```python
from build123d import *

# Parameters (mm, degrees)
BRICK_BODY_PROFILE_W         = 31.8
BRICK_BODY_PROFILE_H         = 15.8
BRICK_BODY_DEPTH             = 9.6
STUDS_PROFILE_2X4_4_8_R      = 2.4
STUDS_8X_4_8_DEPTH           = 1.8
UNDERSIDE_CAVITY_DEPTH       = 22.099289088
UNDERSIDE_CAVITY_DEPTH_BACK  = 7.5
UNDERSIDE_CAVITY_PROFILE_R   = 3.25
UNDERSIDE_CAVITY_PROFILE_R_2 = 2.65


with BuildPart() as part:
    # Brick Body Profile → Brick Body (new body)
    with BuildSketch(Plane.XY):
        Rectangle(BRICK_BODY_PROFILE_W, BRICK_BODY_PROFILE_H)
    extrude(amount=BRICK_BODY_DEPTH)

    # Studs Profile 2x4 Ø4.8 → Studs 8xØ4.8 (add)
    with BuildSketch(Plane.XY.offset(9.6)):
        with Locations((-12, 4)):
            Circle(STUDS_PROFILE_2X4_4_8_R)
        with Locations((-4, 4)):
            Circle(STUDS_PROFILE_2X4_4_8_R)
        with Locations((4, 4)):
            Circle(STUDS_PROFILE_2X4_4_8_R)
        with Locations((12, 4)):
            Circle(STUDS_PROFILE_2X4_4_8_R)
        with Locations(Location((12, -4, 0), (0, 0, 180))):
            Circle(STUDS_PROFILE_2X4_4_8_R)
        with Locations(Location((4, -4, 0), (0, 0, 180))):
            Circle(STUDS_PROFILE_2X4_4_8_R)
        with Locations(Location((-4, -4, 0), (0, 0, 180))):
            Circle(STUDS_PROFILE_2X4_4_8_R)
        with Locations(Location((-12, -4, 0), (0, 0, 180))):
            Circle(STUDS_PROFILE_2X4_4_8_R)
    extrude(amount=STUDS_8X_4_8_DEPTH)

    # Underside Cavity Profile → Underside Cavity (cut, two sides: drawn at the far end of the back side and taken through both)
    # profile 1 of 3: a face of its own
    with BuildSketch(Plane(origin=(0, 0, 0), x_dir=(-1, 0, 0), z_dir=(0, 0, -1)).offset(-UNDERSIDE_CAVITY_DEPTH_BACK)):
        with Locations(Location((-8, 0, 0), (0, 0, 180))):
            Circle(UNDERSIDE_CAVITY_PROFILE_R)
        with Locations(Location((-8, 0, 0), (0, 0, 180))):
            Circle(UNDERSIDE_CAVITY_PROFILE_R_2, mode=Mode.SUBTRACT)
    # profile 2 of 3: a face of its own
    with BuildSketch(Plane(origin=(0, 0, 0), x_dir=(-1, 0, 0), z_dir=(0, 0, -1)).offset(-UNDERSIDE_CAVITY_DEPTH_BACK)):
        with Locations(Location((0, 0, 0), (0, 0, 180))):
            Circle(UNDERSIDE_CAVITY_PROFILE_R)
        with Locations(Location((0, 0, 0), (0, 0, 180))):
            Circle(UNDERSIDE_CAVITY_PROFILE_R_2, mode=Mode.SUBTRACT)
    # profile 3 of 3: a face of its own
    with BuildSketch(Plane(origin=(0, 0, 0), x_dir=(-1, 0, 0), z_dir=(0, 0, -1)).offset(-UNDERSIDE_CAVITY_DEPTH_BACK)):
        with Locations(Location((8, 0, 0), (0, 0, 180))):
            Circle(UNDERSIDE_CAVITY_PROFILE_R)
        with Locations(Location((8, 0, 0), (0, 0, 180))):
            Circle(UNDERSIDE_CAVITY_PROFILE_R_2, mode=Mode.SUBTRACT)
    extrude(amount=UNDERSIDE_CAVITY_DEPTH + UNDERSIDE_CAVITY_DEPTH_BACK, mode=Mode.SUBTRACT)


solid = part.part
```
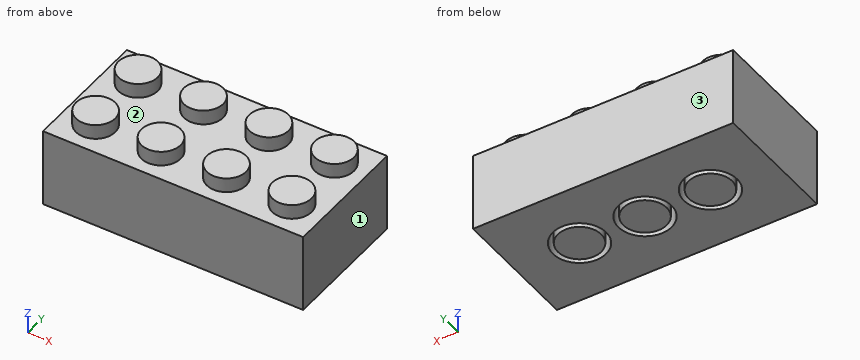
Part model, mm, in its own coordinate system. Face numbers are marked on the shaded views. Round coordinates to 2 decimals unless told otherwise and drop trailing zeros. Write each loop counter-clockwise with the first axis right and the second up, starting at its lowest first coordinate (ties: lowest second). Pieces come first, ordered by that corner, then holes. Notation, with made-up numbers: M -35,8.5 L -25,8.5 A18 ccw -25,38.5 Z; hole C -10,28 d6. An arc over 180 degrees is marked long. One line per question, with ' | ' between items.
(1) Pin check, flat tips, straight feed: pin 1 (4 mm diameter, centred on x = -8, y = 0, fed in from -Z); pin 2 (4 mm diameter, centred on x = 0, y = 0, fed in from +Z). Stop position of each tip, or through.
Answer key:
pin 1: stops at z = 0 | pin 2: stops at z = 9.6
(2) Saw through at C-C on x = 8. Write the cut outline in (y, z).
Answer key:
outline: M -7.9,0 L -3.25,0 L -3.25,7.5 L -2.65,7.5 L -2.65,0 L 2.65,0 L 2.65,7.5 L 3.25,7.5 L 3.25,0 L 7.9,0 L 7.9,9.6 L -7.9,9.6 Z
(3) Saw through at D-D on y = 0. Write the cut outline in (x, z).
Answer key:
outline: M -15.9,0 L -11.25,0 L -11.25,7.5 L -10.65,7.5 L -10.65,0 L -5.35,0 L -5.35,7.5 L -4.75,7.5 L -4.75,0 L -3.25,0 L -3.25,7.5 L -2.65,7.5 L -2.65,0 L 2.65,0 L 2.65,7.5 L 3.25,7.5 L 3.25,0 L 4.75,0 L 4.75,7.5 L 5.35,7.5 L 5.35,0 L 10.65,0 L 10.65,7.5 L 11.25,7.5 L 11.25,0 L 15.9,0 L 15.9,9.6 L -15.9,9.6 Z
(4) Probe line 1 along Y through (x, z) = (-8, 2.25); line 2 along Y through (x, z) = (-10, 3.25); line 3 along Z through (x, y) = (8, -2). List the from-to ranges inside material, lowest first.
Answer key:
line 1: y = -7.9 to -3.25, -2.65 to 2.65, 3.25 to 7.9 | line 2: y = -7.9 to -2.56, -1.74 to 1.74, 2.56 to 7.9 | line 3: z = 0 to 9.6
(5) Saw through at B-B on y = -4. Write the cut outline in (x, z), then the cut area to 3 significant figures.
Answer key:
outline: M -15.9,0 L 15.9,0 L 15.9,9.6 L 14.4,9.6 L 14.4,11.4 L 9.6,11.4 L 9.6,9.6 L 6.4,9.6 L 6.4,11.4 L 1.6,11.4 L 1.6,9.6 L -1.6,9.6 L -1.6,11.4 L -6.4,11.4 L -6.4,9.6 L -9.6,9.6 L -9.6,11.4 L -14.4,11.4 L -14.4,9.6 L -15.9,9.6 Z | area: 340 mm^2
(6) Two-plate mould, pull along Y, no slides. Class the marked faces 1, 2 and 3: released by +Y, released by -Y, zero draft, split by the parting line, or undercut.
Answer key:
face 1: zero draft | face 2: undercut | face 3: released by +Y
(7) Saw through at A-A on z = 6.5. Write the cut outline in (x, y), then the cut area to 3 significant figures.
Answer key:
outline: M -15.9,-7.9 L 15.9,-7.9 L 15.9,7.9 L -15.9,7.9 Z; C -8,0 d5.3; C 0,0 d5.3; C 8,0 d5.3; hole C -8,0 d6.5; hole C 0,0 d6.5; hole C 8,0 d6.5 | area: 469 mm^2
